```python
from build123d import *

# Parameters (mm, degrees)
BOSS_EXTRUDE1_DEPTH     = 3
SKETCH3_R               = 16
CUT_EXTRUDE1_DEPTH      = 1.5
CUT_EXTRUDE2_DEPTH      = 61.827729708
CUT_EXTRUDE2_DEPTH_BACK = 61.827729708
SKETCH4_R               = 4
SKETCH4_R_2             = 3
CHAMFER1_SIZE           = 0.5
FILLET1_R               = 10


with BuildPart() as part:
    # Sketch1 → Boss-Extrude1 (new, symmetric)
    with BuildSketch(Plane.XY):
        with BuildLine():
            Line((50, 6), (5.291502622, 6))
            ThreePointArc((5.291502622, 6), (0, 8), (-5.291502622, 6))
            Line((-5.291502622, 6), (-29.18544931, 6))
            Line((-29.18544931, 6), (-38.257859313, 13.216520767))
            ThreePointArc((-38.257859313, 13.216520767), (-40.615194579, 14.246112449), (-43.172428892, 13.967470655))
            Line((-43.172428892, 13.967470655), (-57.671397892, 8.365596269))
            ThreePointArc((-57.671397892, 8.365596269), (-58.600083665, 7.631017879), (-58.950599334, 6.5))
            Line((-58.950599334, 6.5), (-41.5, 6.5))
            ThreePointArc((-41.5, 6.5), (-37.964466094, 5.035533906), (-36.5, 1.5))
            Line((-36.5, 1.5), (-36.5, -1.5))
            ThreePointArc((-36.5, -1.5), (-37.964466094, -5.035533906), (-41.5, -6.5))
            Line((-41.5, -6.5), (-58.950599334, -6.5))
            ThreePointArc((-58.950599334, -6.5), (-58.600083665, -7.631017879), (-57.671397892, -8.365596269))
            Line((-57.671397892, -8.365596269), (-43.172428892, -13.967470655))
            ThreePointArc((-43.172428892, -13.967470655), (-40.615194579, -14.246112449), (-38.257859313, -13.216520767))
            Line((-38.257859313, -13.216520767), (-29.18544931, -6))
            Line((-29.18544931, -6), (-5.291502622, -6))
            ThreePointArc((-5.291502622, -6), (0, -8), (5.291502622, -6))
            Line((5.291502622, -6), (50, -6))
            ThreePointArc((50, -6), (56, 0), (50, 6))
        make_face()
    extrude(amount=BOSS_EXTRUDE1_DEPTH, both=True)

    # Sketch3 → Cut-Extrude1 (cut)
    with BuildSketch(Plane.XY.offset(3)):
        with Locations((50, 0)):
            Circle(SKETCH3_R)
    cut_extrude1 = extrude(amount=-CUT_EXTRUDE1_DEPTH, mode=Mode.SUBTRACT)

    # Mirror1: Cut-Extrude1 across plane
    add(cut_extrude1.mirror(Plane.XY), mode=Mode.SUBTRACT)

    # Sketch4 → Cut-Extrude2 (cut, two sides: drawn at the far end of the back side and taken through both)
    with BuildSketch(Plane.XY.offset(1.5).offset(-CUT_EXTRUDE2_DEPTH_BACK)):
        with Locations((50, 0)):
            Circle(SKETCH4_R)
        Circle(SKETCH4_R_2)
    extrude(amount=CUT_EXTRUDE2_DEPTH + CUT_EXTRUDE2_DEPTH_BACK, mode=Mode.SUBTRACT)

    # Chamfer1
    chamfer1_edges = [part.edges().sort_by_distance(p)[0] for p in [
        (46, 0, 1.5),
        (46, 0, -1.5),
        (-3, 0, -3),
        (-3, 0, 3),
    ]]
    chamfer(chamfer1_edges, length=CHAMFER1_SIZE)

    # Fillet1
    fillet1_edges = [part.edges().sort_by_distance(p)[0] for p in [
        (-29.18544931, 6, 0),
        (-29.18544931, -6, 0),
    ]]
    fillet(fillet1_edges, radius=FILLET1_R)


solid = part.part
```
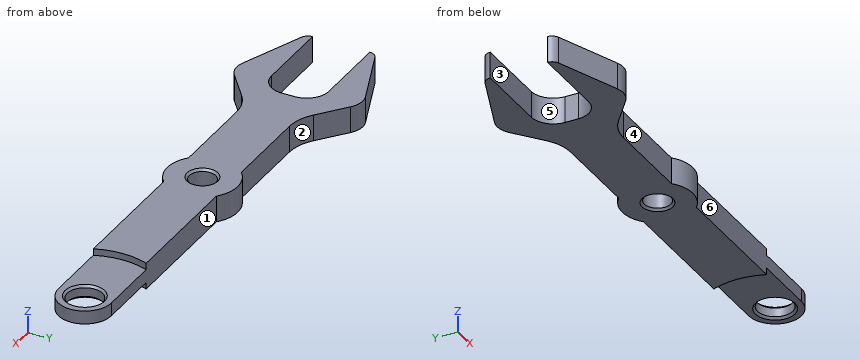
CAD build for the part. Positions are in the model's coordinates, mm. Face numbers are marked on the shaded views. A direction names the side the tool comes from. Round coordinates to 2 decimals unless told otherwise and drop trailing zeros. Write each loop counter-clockwise with the first axis right and the second up, starting at its lowest first coordinate (ties: lowest second). Pieces come first, ordered by that corner, then holes.
Item 1: Band-saw the part on C-C on x = 42.5. Write the cut outline in (y, z), then the cut area to 3 significant figures.
Filled in:
outline: (-6, -1.5) - (6, -1.5) - (6, 1.5) - (-6, 1.5) - close
area: 36.0 mm2
Item 2: Band-saw the part on A-A on y = 0. Write the cut outline in (x, z), then the cut area to 3 significant figures.
Filled in:
outline: (-36.5, -3) - (-3.5, -3) - (-3, -2.5) - (-3, 2.5) - (-3.5, 3) - (-36.5, 3) - close; (3, -2.5) - (3.5, -3) - (34, -3) - (34, -1.5) - (45.5, -1.5) - (46, -1) - (46, 1) - (45.5, 1.5) - (34, 1.5) - (34, 3) - (3.5, 3) - (3, 2.5) - close; (54, -1) - (54.5, -1.5) - (56, -1.5) - (56, 1.5) - (54.5, 1.5) - (54, 1) - close
area: 428 mm2
Item 3: Band-saw the part on D-D on y = 11.25. Write the cut outline in (x, z).
Filled in:
outline: (-50.21, -3) - (-35.79, -3) - (-35.79, 3) - (-50.21, 3) - close
Item 4: Band-saw the part on B-B on x = 0. Write the cut outline in (y, z), then the cut area to 3 significant figures.
Filled in:
outline: (-8, -3) - (-3.5, -3) - (-3, -2.5) - (-3, 2.5) - (-3.5, 3) - (-8, 3) - close; (3, -2.5) - (3.5, -3) - (8, -3) - (8, 3) - (3.5, 3) - (3, 2.5) - close
area: 59.5 mm2
Item 5: Drill centre lines: L1, parallel to X at y = 0, z = -0.4; L2, parallel to X at y = 1.5, z = 0.55; L3, parallel to Y at x = 50, z = -0.35. Where is each one in solid material? Low to high.
Filled in:
L1: x = -36.5 to -3, 3 to 46, 54 to 56
L2: x = -36.5 to -2.6, 2.6 to 46.29, 53.71 to 55.81
L3: y = -6 to -4, 4 to 6
Item 6: Mould opens along X. For the marked faces 4, 5 and 6 say: released by +X, released by -X, zero draft, split by the parting line, or undercut.
Filled in:
face 4: undercut
face 5: released by -X
face 6: zero draft
Item 7: Tool access for the marked faces 1, 2 and 3: list every direction of +Z, -Z, +X, -X, +Y, -Y with a clear straight run to the whole face (end or side of a thin tool).
Filled in:
face 1: +Z, -Z, +X, +Y
face 2: +Z, -Z, +Y
face 3: +Z, -Z, -X
Item 8: Drop flat-ended pins along their axis: pin 1 Ø8 at (x, y) = (0, 0) entering from +Z; pin 2 Ø4 at (x, y) = (38.5, -6) entering from +Z; pin 3 Ø1.8 at (x, z) = (-14.5, -1) entering from +Y; pin 4 Ø1.8 at (x, z) = (-10.5, 1.5) entering from -Y. Give the stop position or say it passes through.
Filled in:
pin 1: stops at z = 3
pin 2: stops at z = 1.5
pin 3: stops at y = 6
pin 4: stops at y = -6
